from build123d import *

# Parameters (mm, degrees)
BASE_BLOCK_SKETCH_R  = 20
BASE_BLOCK_DEPTH     = 32
PIVOT_BOSS_SKETCH_R  = 8
PIVOT_BOSS_DEPTH     = 22
ARM_START            = 20
ARM_PROFILE_SKETCH_R = 8
ARM_1_DEPTH          = 18
ARM_START_2          = -38
SKETCH3_2_R          = 8
ARM_2_DEPTH          = 18
SIDE_LUG_SKETCH_W    = 4
SIDE_LUG_SKETCH_H    = 48
SIDE_LUGS_DEPTH      = 14


with BuildPart() as part:
    # Base Block Sketch → Base Block (new body)
    with BuildSketch(Plane(origin=(0, 0, 0), x_dir=(0, 0, -1), z_dir=(1, 0, 0))):
        with BuildLine():
            Line((-38, 0), (-38, -36))
            Line((-38, -36), (38, -36))
            Line((38, -36), (38, 0))
            ThreePointArc((38, 0), (0, 38), (-38, 0))
        make_face()
        Circle(BASE_BLOCK_SKETCH_R, mode=Mode.SUBTRACT)
    extrude(amount=BASE_BLOCK_DEPTH)

    # Pivot Boss Sketch → Pivot Boss (add)
    # profile 1 of 2: a face of its own
    with BuildSketch(Plane(origin=(0, 0, 0), x_dir=(0, 0, -1), z_dir=(1, 0, 0))):
        with BuildLine():
            Line((-38, -0.287187079), (-38, -84))
            Line((-38, -84), (-70, -84))
            Line((-70, -84), (-70, -28))
            ThreePointArc((-70, -28), (-47.66969722, -21.453197567), (-38, -0.287187079))
        make_face()
        with Locations((-54, -42)):
            Circle(PIVOT_BOSS_SKETCH_R, mode=Mode.SUBTRACT)
        with Locations((-54, -70)):
            Circle(PIVOT_BOSS_SKETCH_R, mode=Mode.SUBTRACT)
    # profile 2 of 2: a face of its own
    with BuildSketch(Plane(origin=(0, 0, 0), x_dir=(0, 0, -1), z_dir=(1, 0, 0))):
        with BuildLine():
            Line((70, -28), (70, -84))
            Line((70, -84), (38, -84))
            Line((38, -84), (38, -0.287187079))
            ThreePointArc((38, -0.287187079), (47.66969722, -21.453197567), (70, -28))
        make_face()
        with Locations(Location((54, -70, 0), (0, 0, 180))):
            Circle(PIVOT_BOSS_SKETCH_R, mode=Mode.SUBTRACT)
        with Locations(Location((54, -42, 0), (0, 0, 180))):
            Circle(PIVOT_BOSS_SKETCH_R, mode=Mode.SUBTRACT)
    extrude(amount=PIVOT_BOSS_DEPTH)

    # Arm Profile Sketch → Arm 1 (add)
    with BuildSketch(Plane.XY.offset(ARM_START)):
        with BuildLine():
            Line((0, -84), (82, -84))
            ThreePointArc((82, -84), (97.824601816, -70.362620868), (86.673441811, -52.697747171))
            Line((86.673441811, -52.697747171), (32, -36))
            Line((32, -36), (0, -36))
            Line((0, -36), (0, -84))
        make_face()
        with Locations((82, -68)):
            Circle(ARM_PROFILE_SKETCH_R, mode=Mode.SUBTRACT)
    extrude(amount=ARM_1_DEPTH)

    # Sketch3_2 → Arm 2 (add)
    with BuildSketch(Plane.XY.offset(ARM_START_2)):
        with BuildLine():
            Line((0, -84), (82, -84))
            ThreePointArc((82, -84), (97.824601816, -70.362620868), (86.673441811, -52.697747171))
            Line((86.673441811, -52.697747171), (32, -36))
            Line((32, -36), (0, -36))
            Line((0, -36), (0, -84))
        make_face()
        with Locations((82, -68)):
            Circle(SKETCH3_2_R, mode=Mode.SUBTRACT)
    extrude(amount=ARM_2_DEPTH)

    # Side Lug Sketch → Side Lugs (add)
    with BuildSketch(Plane.ZY):
        with Locations((-18, -60)):
            Rectangle(SIDE_LUG_SKETCH_W, SIDE_LUG_SKETCH_H)
        with Locations((18, -60)):
            Rectangle(SIDE_LUG_SKETCH_W, SIDE_LUG_SKETCH_H)
    extrude(amount=-SIDE_LUGS_DEPTH)


solid = part.part
CAD build for the part. Positions are in the model's coordinates, mm. A direction names the side the tool comes from. Coordinates: 2 decimals unless noted, no trailing zeros. Write each loop counter-clockwise with the first axis right and the second up, starting at its lowest first coordinate (ties: lowest second). Pieces come first, ordered by that corner, then holes. Notation, with made-up numbers: M 68.5,65 L 87.5,65 A22 ccw 87.5,102 Z; hole C 80,17.5 d10. An arc over 180 degrees is marked long. Return JSON: item names as keys, results as strings.
Item 1: Which spindle directions (+Z, -Z, +X, -X, +Y, -Y) get a long thin tool onto all of the face, cutting with end or side? Do faces 4 (the flat face through (46, -60, -20)), 5 (the flat face through (7, -60, 16)), 6 (the flat face through (32, -23, 1)). Say none if no direction does.
Findings below:
{"face 4": "+X, -Y", "face 5": "+X, -X, -Y", "face 6": "+Z, -Z, +X, +Y"}
Item 2: Slice it at D-D, the plane x = 41.5. Write the cut outline in (y, z).
Findings below:
{"outline": "M -84,-38 L -38.9,-38 L -38.9,-20 L -84,-20 Z; M -84,20 L -38.9,20 L -38.9,38 L -84,38 Z"}
Item 3: Drop flat-ended pins along their axis: pin 1 Ø21 at (y, z) = (-42, -54) entering from +X; pin 2 Ø3 at (x, y) = (12, 7) entering from -Z; pin 3 Ø24 at (x, y) = (72, -66) entering from -Z. Give the stop position or say it passes through.
Findings below:
{"pin 1": "stops at x = 22", "pin 2": "stops at z = -37.6", "pin 3": "stops at z = -38"}
Item 4: Slice it at C-C, the plane z = -54. Write the cut outline in (x, y), and give its area (3 significant figures).
Findings below:
{"outline": "M 0,-84 L 22,-84 L 22,-78 L 0,-78 Z; M 0,-62 L 22,-62 L 22,-50 L 0,-50 Z; M 0,-34 L 22,-34 L 22,-25.59 L 0,-25.59 Z", "area": "581 mm2"}
Item 5: Slice it at A-A, the plane y = -58. Write the cut outline in (x, z), and give its area (3 significant figures).
Findings below:
{"outline": "M 0,-70 L 22,-70 L 22,-38 L 94.49,-38 L 94.49,-20 L 14,-20 L 14,-16 L 0,-16 Z; M 0,16 L 14,16 L 14,20 L 94.49,20 L 94.49,38 L 22,38 L 22,70 L 0,70 Z", "area": "4,920 mm2"}
Item 6: Probe line 1 (Z direction, x = 30, y = -43); line 2 (Y direction, x = 5.25, z = -54); line 3 (Z direction, x = 12, y = -35.5). List the from-to ranges inside material, lowest first. Write a range as from..to.
Findings below:
{"line 1": "z = -38..-20, 20..38", "line 2": "y = -84..-78, -62..-50, -34..-25.59", "line 3": "z = -70..-58.66, -49.34..49.34, 58.66..70"}
Item 7: Two-plate mould, pull along X, no slides. Class faces 1 (the cylindrical face through (80.959, -60.068, 28.874)), 2 (the flat face through (14, -60, -18)), 3 (the cylindrical face through (15.78, 37.99, -0.84)): +X half, -X half, draft (parallel to the pull), parting line (faces both ways), or undercut.
Findings below:
{"face 1": "undercut", "face 2": "+X half", "face 3": "draft"}
Item 8: Slice it at B-B, the plane z = 0. Write the cut outline in (x, y), and give its area (3 significant figures).
Findings below:
{"outline": "M 0,-36 L 32,-36 L 32,-20 L 0,-20 Z; M 0,20 L 32,20 L 32,38 L 0,38 Z", "area": "1,090 mm2"}
